Read the model definition and answer for the solid it produces. Units are mm, in the model's axes. A direction names the side the tool comes from. Round coordinates to 2 decimals unless told otherwise and drop trailing zeros. Loops run counter-clockwise (first coordinate to the right, second up) from the corner with the lowest first, then second, coordinate; pieces in that order, holes last. Notation, with made-up numbers: M -3,-15 L 37,-15 A20 cw 37,-9 Z; hole C 52.5,78 d2. An arc over 180 degrees is marked long. Write each question's results on one line, items separated by ' | '.
from build123d import *

# Parameters (mm, degrees)
MOUNTING_PLATE_SKETCH_R         = 15
MOUNTING_PLATE_SKETCH_R_2       = 10
MOUNTING_PLATE_SKETCH_R_3       = 45
MOUNTING_PLATE_SKETCH_R_4       = 28
MOUNTING_PLATE_200X130X20_DEPTH = 20
PIVOT_LUG_SKETCH_R              = 10
PIVOT_LUG_DEPTH                 = 15
RING_BOSS_SKETCH_R              = 28
RING_BOSS_SKETCH_R_2            = 20
RING_BOSS_6MM_DEPTH             = 6


with BuildPart() as part:
    # Shaft Profile Sketch → Grooved Shaft Revolve (revolve)
    with BuildSketch(Plane.XY):
        Polygon((-45, 57.5), (-45, -22.5), (-40, -22.5), (-40, -32.5), (-45, -32.5), (-45, -57.5), (-20, -57.5), (-20, 57.5), align=None)
    revolve(axis=Axis((0, 146.177983413, 0), (0, -1, 0)))

    # Mounting Plate Sketch → Mounting Plate 200x130x20 (add)
    # profile 1 of 2: a face of its own
    with BuildSketch(Plane(origin=(0, 57.5, 0), x_dir=(1, 0, 0), z_dir=(0, 1, 0))):
        with BuildLine():
            ThreePointArc((85, 65), (95.606601718, 60.606601718), (100, 50))
            Line((100, 50), (100, -50))
            ThreePointArc((100, -50), (95.606601718, -60.606601718), (85, -65))
            Line((85, -65), (-85, -65))
            ThreePointArc((-85, -65), (-95.606601718, -60.606601718), (-100, -50))
            Line((-100, -50), (-100, 50))
            ThreePointArc((-100, 50), (-95.606601718, 60.606601718), (-85, 65))
            Line((-85, 65), (85, 65))
        make_face()
        with Locations(Location((70, 35, 0), (0, 0, 180))):
            Circle(MOUNTING_PLATE_SKETCH_R, mode=Mode.SUBTRACT)
        with Locations(Location((70, -35, 0), (0, 0, 180))):
            Circle(MOUNTING_PLATE_SKETCH_R, mode=Mode.SUBTRACT)
        with Locations(Location((-70, 0, 0), (0, 0, 180))):
            Circle(MOUNTING_PLATE_SKETCH_R_2, mode=Mode.SUBTRACT)
        with Locations(Location((-70, -35, 0), (0, 0, 180))):
            Circle(MOUNTING_PLATE_SKETCH_R, mode=Mode.SUBTRACT)
        with Locations(Location((-70, 35, 0), (0, 0, 180))):
            Circle(MOUNTING_PLATE_SKETCH_R, mode=Mode.SUBTRACT)
        with Locations(Location((70, 0, 0), (0, 0, 180))):
            Circle(MOUNTING_PLATE_SKETCH_R_2, mode=Mode.SUBTRACT)
        with Locations(Location((0, 0, 0), (0, 0, 180))):
            Circle(MOUNTING_PLATE_SKETCH_R_3, mode=Mode.SUBTRACT)
    # profile 2 of 2: a face of its own
    with BuildSketch(Plane(origin=(0, 57.5, 0), x_dir=(1, 0, 0), z_dir=(0, 1, 0))):
        with Locations(Location((0, 0, 0), (0, 0, 180))):
            Circle(MOUNTING_PLATE_SKETCH_R_3)
        with Locations(Location((0, 0, 0), (0, 0, 180))):
            Circle(MOUNTING_PLATE_SKETCH_R_4, mode=Mode.SUBTRACT)
    extrude(amount=MOUNTING_PLATE_200X130X20_DEPTH)

    # Pivot Lug Sketch → Pivot Lug (add)
    with BuildSketch(Plane.XY.offset(65)):
        with BuildLine():
            Line((15, 97.5), (15, 77.5))
            Line((15, 77.5), (-15, 77.5))
            Line((-15, 77.5), (-15, 97.5))
            ThreePointArc((-15, 97.5), (0, 112.5), (15, 97.5))
        make_face()
        with Locations((0, 97.5)):
            Circle(PIVOT_LUG_SKETCH_R, mode=Mode.SUBTRACT)
    extrude(amount=-PIVOT_LUG_DEPTH)

    # Ring Boss Sketch → Ring Boss 6mm (add)
    with BuildSketch(Plane(origin=(0, 57.5, 0), x_dir=(1, 0, 0), z_dir=(0, 1, 0))):
        with Locations(Location((0, 0, 0), (0, 0, 180))):
            Circle(RING_BOSS_SKETCH_R)
        with Locations(Location((0, 0, 0), (0, 0, 180))):
            Circle(RING_BOSS_SKETCH_R_2, mode=Mode.SUBTRACT)
    extrude(amount=RING_BOSS_6MM_DEPTH)


solid = part.part
Item 1: For faces 5 (the face through (-15, 87, 58)), 6 (the face through (8.67, -27.57, 39.05)), 7 (the face through (0, 87, 50)), 8 (the face through (46, 57.5, -1)), determine the directions among +Z, -Z, +X, -X, +Y, -Y from which every point of the face is accessible in a straight line to the end or side of a thin tool.
Outcome:
face 5: +Z, -Z, -X, +Y | face 6: none | face 7: -Z, +X, -X, +Y | face 8: -Y
Item 2: The mould has two halves that part along Z. Classify faces 1 (the face through (95.72, 67.36, 60.49)), 2 (the face through (80, 67, 0)), 3 (the face through (-20.765, -45.175, 39.923)), 4 (the face through (-100, 67, 1)): pulls with the +Z half, pulls with the -Z half, needs draft (parallel to the pull), parting line crosses it, or undercut.
Outcome:
face 1: pulls with the +Z half | face 2: undercut | face 3: parting line crosses it | face 4: needs draft
Item 3: The part is cut by section A-A (x = 70). Determine the outline of the cut face in (y, z), plus the area to 3 significant figures.
Outcome:
outline: M 57.5,-65 L 77.5,-65 L 77.5,-50 L 57.5,-50 Z; M 57.5,-20 L 77.5,-20 L 77.5,-10 L 57.5,-10 Z; M 57.5,10 L 77.5,10 L 77.5,20 L 57.5,20 Z; M 57.5,50 L 77.5,50 L 77.5,65 L 57.5,65 Z | area: 1,000 mm2
Item 4: Straight lines are drawn through the part: line 1 (Z direction, x = 70, y = 73); line 2 (X direction, y = -10, z = 0); line 3 (Z direction, x = 0, y = -31.5). For each, find the intervals that lie inside material, in ascending order.
Outcome:
line 1: z = -65 to -50, -20 to -10, 10 to 20, 50 to 65 | line 2: x = -45 to -20, 20 to 45 | line 3: z = -40 to -20, 20 to 40
Item 5: The part is cut by section B-B (z = 0). State how many separate pieces and enclosed holes the cut face has, plus the area to 3 significant figures.
Outcome:
separate pieces: 4 | enclosed holes: 0 | area: 7,830 mm2
Item 6: Flat-ended cylindrical pins translate along their axes: pin 1 (18 mm diameter, centred on x = 70, z = -35, fed in from +Y); pin 2 (10 mm diameter, centred on y = -9, z = 32.5, fed in from +X); pin 3 (24 mm diameter, centred on x = 7, y = 97.5, fed in from -Z); pin 4 (8 mm diameter, centred on x = 33.5, z = 16.5, fed in from +Y). Find the tip coordinate at first contact, or state that the pin passes through.
Outcome:
pin 1: passes through | pin 2: stops at x = 35.62 | pin 3: stops at z = 50 | pin 4: stops at y = 77.5
Item 7: The part is cut by section D-D (y = 84). Determine the outline of the cut face in (x, z).
Outcome:
outline: M -15,50 L 15,50 L 15,65 L -15,65 Z
